from build123d import *

# Parameters (mm, degrees)
EXTRUDE_1_DEPTH         = 8
CHAMFER_1_SIZE          = 10
HOLE_WIZARD_16_0_16_1_D = 16


with BuildPart() as part:
    # 草图1 → 凸台-拉伸1 (new body)
    with BuildSketch(Plane(origin=(0, 0, 0), x_dir=(1, 0, 0), z_dir=(0, 1, 0))):
        Polygon((0, 0), (0, 90), (90, 0), align=None)
    extrude(amount=EXTRUDE_1_DEPTH)

    # 倒角1
    chamfer_1_edges = [part.edges().sort_by_distance(p)[0] for p in [
        (0, 4, 0),
    ]]
    chamfer(chamfer_1_edges, length=CHAMFER_1_SIZE)

    # Ø16.0 (16) 直径孔1 (through all)
    with Locations(Plane(origin=(0, 8, 0), x_dir=(1, 0, 0), z_dir=(0, 1, 0))):
        with Locations((25, 25)):
            Hole(HOLE_WIZARD_16_0_16_1_D / 2)


solid = part.part
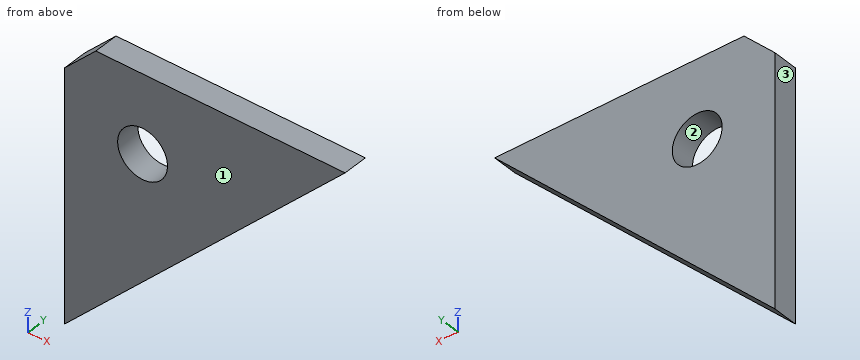
Work out the finished part from the listing and answer in its coordinate system (mm). Face numbers are marked on the shaded views. Give positions to 0.01 mm unless a question says otherwise; leave off trailing zeros. Write each loop counter-clockwise with the first axis right and the second up, starting at its lowest first coordinate (ties: lowest second). Pieces come first, ordered by that corner, then holes.
Q1. For a pull along X with two mould halves and no side action, classify the marked faces 1, 2 and 3 as released by +X, released by -X, zero draft, split by the parting line, or undercut.
Answer:
face 1: zero draft
face 2: undercut
face 3: released by -X
Q2. Given pin 1 (21 mm diameter, centred on x = 25, z = -25, fed in from +Y), flat-ended and moving along its own axis, determine where the tip first touches the part or whether it passes through.
Answer:
pin 1: stops at y = 8
Q3. The part is cut by section D-D on x = 75. Give the vertices of the cut face in (y, z).
Answer:
outline: (0, -15) - (8, -15) - (8, 0) - (0, 0) - close
Q4. The part is cut by section A-A on z = -25. Give the vertices of the cut face in (x, y).
Answer:
outline: (0, 0) - (17, 0) - (17, 8) - (0, 8) - close; (33, 0) - (65, 0) - (65, 8) - (33, 8) - close
Q5. Straight lines are drawn through the part: L1, parallel to Z at x = 25, y = 2.5; L2, parallel to Z at x = 28.5, y = 5; L3, parallel to Z at x = 46, y = 0.75. For each, find the intervals that lie inside material, in ascending order.
Answer:
L1: z = -65 to -33, -17 to 0
L2: z = -61.5 to -32.19, -17.81 to 0
L3: z = -44 to 0
Q6. The part is cut by section B-B on x = 25. Give the vertices of the cut face in (y, z).
Answer:
outline: (0, -65) - (8, -65) - (8, -33) - (0, -33) - close; (0, -17) - (8, -17) - (8, 0) - (0, 0) - close
Q7. The part is cut by section C-C on y = 2. Give the vertices of the cut face in (x, z).
Answer:
outline: (0, -90) - (90, 0) - (10, 0) - (0, -10) - close; hole circle Ø16 at (25, -25)
